The model under review builds one solid part; all positions refer to its coordinate system, in mm. A direction names the side the tool comes from. Round coordinates to 2 decimals unless told otherwise and drop trailing zeros. Loops run counter-clockwise (first coordinate to the right, second up) from the corner with the lowest first, then second, coordinate; pieces in that order, holes last. Notation, with made-up numbers: (-37, 64) -> (-26, 64) arc R24 ccw to (-26, 97) -> close; hole circle Ø2 at (26, -9.5). An arc over 180 degrees is marked (long way). Write each question's results on one line, items separated by ' | '. Start each with the question number.
Item 1: For L1, parallel to Y at x = 0, z = 0.7; L2, parallel to Y at x = 0, z = -3.7; L3, parallel to X at y = 0.5, z = 0.75, list the stretches that pass through material, from the lowest coordinate up. Write a range as from..to.
Item 2: Clearance check with flat-ended pins moving along their axes: pin 1 Ø6 at (x, y) = (0, 0) entering from +Z; pin 2 Ø1.5 at (y, z) = (-5, -0.5) entering from +X; pin 3 Ø2 at (y, z) = (1.5, -1.5) entering from +X. State where each tip first meets the part, or that it passes through.
Item 3: We need section A-A (z = -1.75). Give the boundary of the cut face in (x, y).
Item 4: Tool access review of faces 4 (the flat face through (3, -3, -6.5)), 5 (the cylindrical face through (-5.158, -3.955, 0.592)): name each direction out of +Z, -Z, +X, -X, +Y, -Y from which nothing blocks a thin tool from reaching the whole face with its end or side.
Item 5: Mouldability with a two-part tool opening along X and no side actions: class faces 1 (the flat face through (5.66, 3.2, -3.21)), 2 (the cylindrical face through (-0.74, -3.32, 0.69)), 3 (the flat face through (3, -3, 1.4)) as pulls with the +X half, pulls with the -X half, needs draft (parallel to the pull), parting line crosses it, or undercut.
from build123d import *
from OCP.BRepFilletAPI import BRepFilletAPI_MakeChamfer

# Parameters (mm, degrees)
SKETCH1_R        = 3.3235
BASENUT_DEPTH    = 6.5
ENDCHAMFER_SIZE  = 0.4
ENDCHAMFER_SIZE2 = 0.230940108
SKETCH_1_R       = 6.5
SKETCH_1_R_2     = 3.4
EXTRUDE_1_DEPTH  = 1.4
CHAMFER_1_SIZE   = 0.2


with BuildPart() as part:
    # Sketch1 → BaseNut (new body)
    with BuildSketch(Plane.XY):
        Polygon((3.75277675, -6.5), (7.505553499, 0), (3.75277675, 6.5), (-3.75277675, 6.5), (-7.505553499, 0), (-3.75277675, -6.5), align=None)
        Circle(SKETCH1_R, mode=Mode.SUBTRACT)
    extrude(amount=-BASENUT_DEPTH)

    # Sketch2 → Double-Chamfer (revolve, cut)
    with BuildSketch(Plane(origin=(0, 0, 0), x_dir=(1, 0, 0), z_dir=(0, 1, 0))):
        Polygon((-7.505553499, 6.5), (-6.125, 6.5), (-7.505553499, 5.702937065), align=None)
        Polygon((-7.505553499, 0.797062935), (-7.505553499, 0), (-6.125, 0), align=None)
    revolve(axis=Axis((0, 0, -3.375940562), (0, 0, 1)), mode=Mode.SUBTRACT)

    # EndChamfer: one chamfer whose edges measure the first distance from different faces: ONE call of the kernel's chamfer builder (chamfer() names one face for all edges)
    endchamfer_edges_1 = [part.edges().sort_by_distance(p)[0] for p in [
        (-3.3235, 0, -6.5),
    ]]
    endchamfer_side_1 = [part.faces().sort_by_distance(p)[0] for p in [
        (-3.3235, 0, -3.25),
    ]]
    endchamfer_edges_2 = [part.edges().sort_by_distance(p)[0] for p in [
        (-3.3235, 0, 0),
    ]]
    endchamfer_side_2 = [part.faces().sort_by_distance(p)[0] for p in [
        (5.951758839, 0, 0),
    ]]
    endchamfer = BRepFilletAPI_MakeChamfer(part.part.solid().wrapped)
    for e in endchamfer_edges_1:
        endchamfer.Add(ENDCHAMFER_SIZE, ENDCHAMFER_SIZE2, e.wrapped, endchamfer_side_1[0].wrapped)  # the first distance lies on this face
    for e in endchamfer_edges_2:
        endchamfer.Add(ENDCHAMFER_SIZE, ENDCHAMFER_SIZE2, e.wrapped, endchamfer_side_2[0].wrapped)  # the first distance lies on this face
    add(Compound.cast(endchamfer.Shape()), mode=Mode.REPLACE)

    # 草图1 → 凸台-拉伸1 (add)
    with BuildSketch(Plane.XY):
        Circle(SKETCH_1_R)
        Circle(SKETCH_1_R_2, mode=Mode.SUBTRACT)
    extrude(amount=EXTRUDE_1_DEPTH)

    # 倒角1
    chamfer_1_edges = [part.edges().sort_by_distance(p)[0] for p in [
        (-6.5, 0, 1.4),
    ]]
    chamfer(chamfer_1_edges, length=CHAMFER_1_SIZE)


solid = part.part
Here are the results:
1) L1: y = -6.5..-3.4, 3.4..6.5 | L2: y = -6.5..-3.32, 3.32..6.5 | L3: x = -6.48..-3.36, 3.36..6.48
2) pin 1: passes through | pin 2: stops at x = 5.05 | pin 3: stops at x = 7.22
3) outline: (-7.51, 0) -> (-3.75, -6.5) -> (3.75, -6.5) -> (7.51, 0) -> (3.75, 6.5) -> (-3.75, 6.5) -> close; hole circle Ø6.65 at (0, 0)
4) face 4: -Z, +X, -X, +Y, -Y | face 5: +Z
5) face 1: pulls with the +X half | face 2: undercut | face 3: needs draft
